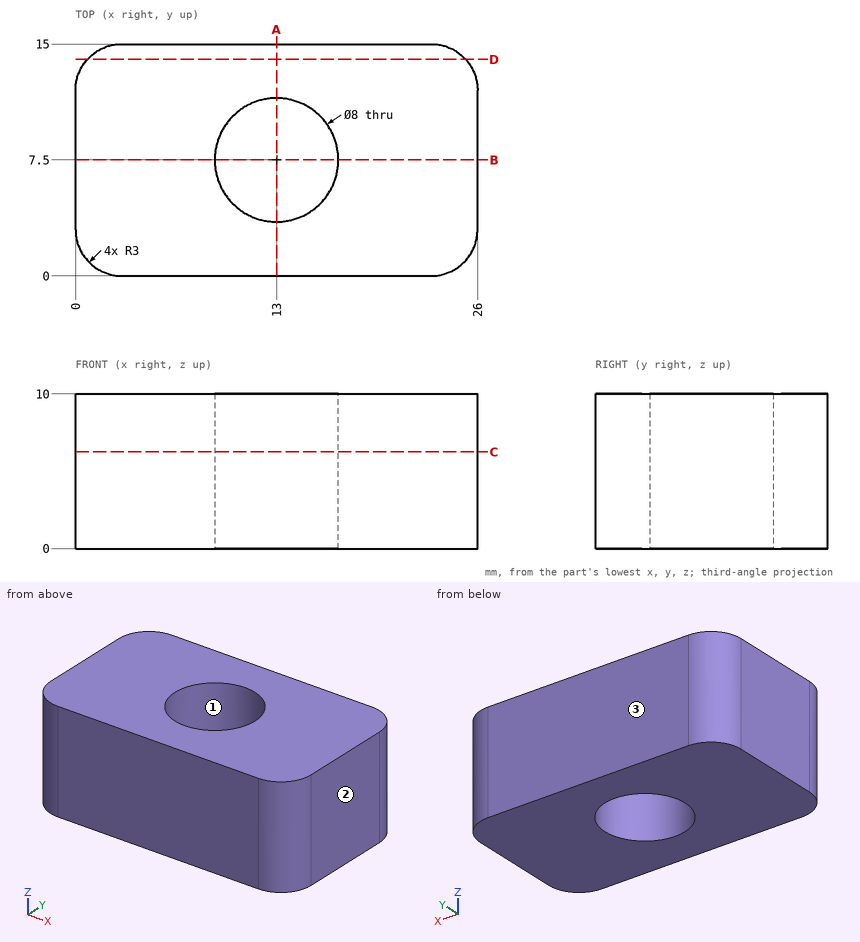
Here's the drawing with two shaded views (mm, measured from the low corner). I have some questions. Give positions to 0.01 mm unless a question says otherwise; leave off trailing zeros. Loops run counter-clockwise (first coordinate to the right, second up) from the corner with the lowest first, then second, coordinate; pieces in that order, holes last. Notation, with made-up numbers: (50, 47) - (83, 47) arc R15 cw to (83, 68) - close; hole circle Ø9 at (10, 20). An arc over 180 degrees is marked (long way). One line per item, written item: value.
(1) If we section it at B-B, the plane y = 7.5: List the corners of the cut face in (x, z) for me.
Verdict:
outline: (0, 0) - (9, 0) - (9, 10) - (0, 10) - close; (17, 0) - (26, 0) - (26, 10) - (17, 10) - close
(2) If we section it at C-C, the plane z = 6.25: List the corners of the cut face in (x, y) for me.
Verdict:
outline: (0, 3) arc R3 ccw to (3, 0) - (23, 0) arc R3 ccw to (26, 3) - (26, 12) arc R3 ccw to (23, 15) - (3, 15) arc R3 ccw to (0, 12) - close; hole circle Ø8 at (13, 7.5)
(3) If we section it at A-A, the plane x = 13: List the corners of the cut face in (y, z) for me.
Verdict:
outline: (0, 0) - (3.5, 0) - (3.5, 10) - (0, 10) - close; (11.5, 0) - (15, 0) - (15, 10) - (11.5, 10) - close
(4) If we mould it in two halves opening along X, with no side actions, what happens to the marked faces 1, 2 and 3? For each: released by +X, released by -X, zero draft, split by the parting line, or undercut.
Verdict:
face 1: undercut
face 2: released by +X
face 3: zero draft
(5) I'm going to push flat-ended pins straight in: pin 1 (6 mm diameter, centred on x = 12.5, y = 10.5, fed in from -Z); pin 2 (5 mm diameter, centred on x = 13, y = 7.5, fed in from -Z). Where does each tip first touch, or does it pass through?
Verdict:
pin 1: z = 0
pin 2: through
(6) If we section it at D-D, the plane y = 14: List the corners of the cut face in (x, z) for me, plus the area to 3 significant figures.
Verdict:
outline: (0.76, 0) - (25.24, 0) - (25.24, 10) - (0.76, 10) - close
area: 245 mm^2
(7) I need wall thicknesses on line 1 along Y through (x, z) = (13, 5.75); line 2 along Y through (x, z) = (16.25, 9); line 3 along X through (y, z) = (10, 2.25). Which ranges of each line are inside material? Lowest first, please.
Verdict:
line 1: 0 to 3.5, 11.5 to 15
line 2: 0 to 5.17, 9.83 to 15
line 3: 0 to 9.88, 16.12 to 26
